```python
from build123d import *

# Parameters (mm, degrees)
SKETCH1_W                  = 120
SKETCH1_H                  = 90
BOSS_EXTRUDE1_DEPTH        = 10
SKETCH2_R                  = 0.808722662
CUT_EXTRUDE1_DEPTH         = 8
M5_TAPPED_HOLE1_AT_2_COUNT = 2
M5_TAPPED_HOLE1_AT_2_PITCH = 76
SKETCH4_R                  = 1.068128835
SKETCH4_R_2                = 0.756333918
SKETCH4_R_3                = 1.055288756
CUT_EXTRUDE2_DEPTH         = 6.5
M5_TAPPED_HOLE2_D          = 4.2
M5_TAPPED_HOLE2_DEPTH      = 12.4
M5_TAPPED_HOLE2_TIP        = 1.2618073
CUT_EXTRUDE3_DEPTH         = 76.663729812


with BuildPart() as part:
    # Sketch1 → Boss-Extrude1 (new body)
    with BuildSketch(Plane(origin=(0, 0, 0), x_dir=(1, 0, 0), z_dir=(0, 1, 0))):
        Rectangle(SKETCH1_W, SKETCH1_H)
    extrude(amount=BOSS_EXTRUDE1_DEPTH)

    # Sketch2 → Cut-Extrude1 (cut)
    with BuildSketch(Plane.ZY.offset(60)):
        with Locations(Location((-38, 5, 0), (0, 0, 180))):
            Circle(SKETCH2_R)
        with Locations((38, 5)):
            Circle(SKETCH2_R)
    extrude(amount=-CUT_EXTRUDE1_DEPTH, mode=Mode.SUBTRACT)

    # Sketch3 → M5 Tapped Hole1 (revolve, cut)
    with BuildSketch(Plane(origin=(-60, 5, 38), x_dir=(0, 0, 1), z_dir=(0, 1, 0))):
        Polygon((0, 0), (0, 13.6618073), (2.1, 12.4), (2.1, 0), align=None)
    m5_tapped_hole1 = revolve(axis=Axis((-66.35, 5, 38), (1, 0, 0)), mode=Mode.SUBTRACT)

    # M5 Tapped Hole1 at 2: M5 Tapped Hole1 ×2
    with Locations(*[(0, 0, -i * M5_TAPPED_HOLE1_AT_2_PITCH) for i in range(1, M5_TAPPED_HOLE1_AT_2_COUNT)]):
        add(m5_tapped_hole1, mode=Mode.SUBTRACT)

    # Mirror1: M5 Tapped Hole1 across plane
    add(m5_tapped_hole1.mirror(Plane(origin=(0, 0, 0), x_dir=(0, 0, 1), z_dir=(1, 0, 0))), mode=Mode.SUBTRACT)

    # Mirror1 copy 1 sketch → Mirror1 copy 1 (revolve, cut)
    with BuildSketch(Plane(origin=(60, 5, -38), x_dir=(0, 0, 1), z_dir=(0, 1, 0))):
        Polygon((0, 0), (0, -13.6618073), (2.1, -12.4), (2.1, 0), align=None)
    revolve(axis=Axis((66.35, 5, -38), (1, 0, 0)), mode=Mode.SUBTRACT)

    # Sketch4 → Cut-Extrude2 (cut)
    with BuildSketch(Plane.XY.offset(45)):
        with Locations((45, 5)):
            Circle(SKETCH4_R)
        with Locations((0, 5)):
            Circle(SKETCH4_R_2)
        with Locations((-45, 5)):
            Circle(SKETCH4_R_3)
    extrude(amount=-CUT_EXTRUDE2_DEPTH, mode=Mode.SUBTRACT)

    # M5 Tapped Hole2
    with Locations(Plane(origin=(-45, 5, 45), x_dir=(1, 0, 0), z_dir=(0, 0, 1))):
        with Locations((0, 0), (45, 0), (90, 0)):
            Hole(M5_TAPPED_HOLE2_D / 2, depth=M5_TAPPED_HOLE2_DEPTH)
            with Locations((0, 0, -(M5_TAPPED_HOLE2_DEPTH + M5_TAPPED_HOLE2_TIP / 2))):  # 118° drill point
                Cone(0, M5_TAPPED_HOLE2_D / 2, M5_TAPPED_HOLE2_TIP, mode=Mode.SUBTRACT)

    # Sketch6 → Cut-Extrude3 (cut, through all)
    with BuildSketch(Plane.XZ):
        with BuildLine():
            Line((-35, 30), (35, 30))
            ThreePointArc((35, 30), (38.535533906, 28.535533906), (40, 25))
            Line((40, 25), (40, -25))
            ThreePointArc((40, -25), (38.535533906, -28.535533906), (35, -30))
            Line((35, -30), (-35, -30))
            ThreePointArc((-35, -30), (-38.535533906, -28.535533906), (-40, -25))
            Line((-40, -25), (-40, 25))
            ThreePointArc((-40, 25), (-38.535533906, 28.535533906), (-35, 30))
        make_face()
    extrude(amount=-CUT_EXTRUDE3_DEPTH, mode=Mode.SUBTRACT)


solid = part.part
```
Can you work these out from the model? Positions are in its coordinate system, mm. A direction names the side the tool comes from. Give positions to 0.01 mm unless a question says otherwise; leave off trailing zeros. Order: outer loops, then holes, each group sorted by start corner. A loop starts at its lowest first (then second) coordinate and runs counter-clockwise, first axis right, second up. Notation, with made-up numbers: (17.5, 0.25) - (30.5, 0.25) arc R34 ccw to (30.5, 31.25) - close; hole circle Ø5 at (-5.5, 46). An arc over 180 degrees is marked (long way). Use a Markdown table: item, result. Add a question column.
Q1. If we section it at C-C on y = 1.25: Write out the boundary of the cut face in (x, z).
Q2. Please list where these lines run through material, in increasing order: line 1 along X through (y, z) = (5, 40.5); line 2 along Z through (x, y) = (-50.75, 5); line 3 along Y through (x, z) = (54.75, -38).
Q3. If we section it at B-B on x = -8: Write out the boundary of the cut face in (y, z), plus the area to 3 significant figures.
Q4. I'm going to push flat-ended pins straight in: pin 1 (2.5 mm diameter, centred on y = 5, z = 38, fed in from -X); pin 2 (2.5 mm diameter, centred on x = 0, y = 5, fed in from +Z); pin 3 (3.5 mm diameter, centred on y = 5, z = 38, fed in from -X). Where does each tip first touch, or does it pass through?
Q5. If we section it at A-A on z = 20: Write out the boundary of the cut face in (x, y), plus the area to 3 significant figures.
Q6. If we section it at D-D on z = 38: Write out the boundary of the cut face in (x, y), plus the area to 3 significant figures.
Q7. On a 3-axis mill with a long thin cutter (end or side, diameter ignored), from which of +Z, -Z, +X, -X, +Y, -Y can I reach the whole of each face in a straight line? I mean faces 1 (the conical face through (46.56, 4.75, -38.27)), 2 (the cylindrical face through (39, 5, -28)), 3 (the cylindrical face through (-53.89, 4.91, 35.9)). Say none if no direction works.
Q8. If we mould it in two halves opening along Y, with no side actions, what happens to faces 4 (the cylindrical face through (-38, 5, -29)), 5 (the flat face through (-1, 0, -31)), 6 (the cylindrical face through (53.89, 4.91, -40.1))? For each: released by +Y, released by -Y, zero draft, split by the parting line, or undercut.
Answers follow:
| question | item | result |
|---|---|---|
| 1 | outline | (-60, -45) - (60, -45) - (60, 45) - (-60, 45) - close; hole (-40, -25) arc R5 ccw to (-35, -30) - (35, -30) arc R5 ccw to (40, -25) - (40, 25) arc R5 ccw to (35, 30) - (-35, 30) arc R5 ccw to (-40, 25) - close |
| 2 | line 1 | x = -60 to -47.1, -42.9 to -2.1, 2.1 to 42.9, 47.1 to 60 |
| 2 | line 2 | z = -45 to -40.1, -35.9 to 35.9, 40.1 to 45 |
| 2 | line 3 | y = 0 to 2.9, 7.1 to 10 |
| 3 | outline | (0, -45) - (10, -45) - (10, -30) - (0, -30) - close; (0, 30) - (10, 30) - (10, 45) - (0, 45) - close |
| 3 | area | 300 mm^2 |
| 4 | pin 1 | stops at x = -47.09 |
| 4 | pin 2 | stops at z = 32.09 |
| 4 | pin 3 | stops at x = -47.39 |
| 5 | outline | (-60, 0) - (-40, 0) - (-40, 10) - (-60, 10) - close; (40, 0) - (60, 0) - (60, 10) - (40, 10) - close |
| 5 | area | 400 mm^2 |
| 6 | outline | (-60, 0) - (60, 0) - (60, 2.9) - (47.6, 2.9) - (46.89, 4.08) arc R2.1 cw (long way) to (46.89, 5.92) - (47.6, 7.1) - (60, 7.1) - (60, 10) - (-60, 10) - (-60, 7.1) - (-47.6, 7.1) - (-46.89, 5.92) arc R2.1 cw (long way) to (-46.89, 4.08) - (-47.6, 2.9) - (-60, 2.9) - close; hole circle Ø4.2 at (0, 5) |
| 6 | area | 1,050 mm^2 |
| 7 | face 1 | +X |
| 7 | face 2 | +Y, -Y |
| 7 | face 3 | -X |
| 8 | face 4 | zero draft |
| 8 | face 5 | released by -Y |
| 8 | face 6 | undercut |
